Input: part model. Units: mm. Frame: model coordinates. A direction names the side the tool comes from. Coordinates: 2 decimals unless noted, no trailing zeros. Write each loop counter-clockwise with the first axis right and the second up, starting at its lowest first coordinate (ties: lowest second). Pieces come first, ordered by that corner, then holes. Notation, with made-up numbers: (77, 28) - (86, 28) arc R22 ccw to (86, 46) - close; hole circle Ø4 at (-15.75, 7.5). An arc over 180 degrees is marked (long way). Use CSV: the item, a comma, the result in double quotes.
```python
from build123d import *

# Parameters (mm, degrees)
CHAMFER1_SIZE      = 3
SKETCH2_W          = 4
SKETCH2_H          = 70.381112312
CUT_EXTRUDE2_DEPTH = 228.158534949


with BuildPart() as part:
    # Sketch1 → Revolve1 (revolve)
    with BuildSketch(Plane.XY, mode=Mode.PRIVATE) as revolve1_sk:
        Polygon((0, 115), (36, 115), (36, 112), (51, 112), (51, 120), (151, 120), (151, 103.5), (36, 98.7), (0, 98.7), align=None)
    revolve(revolve1_sk.sketch.rotate(Axis((0, 0, 0), (1, 0, 0)), 90), axis=Axis((0, 0, 0), (1, 0, 0)))

    # Chamfer1
    chamfer1_edges = [part.edges().sort_by_distance(p)[0] for p in [
        (0, 0, -115),
    ]]
    chamfer(chamfer1_edges, length=CHAMFER1_SIZE)

    # Sketch2 → Cut-Extrude2 (cut, through all)
    with BuildSketch(Plane(origin=(0, 0, 0), x_dir=(0, 0, -1), z_dir=(1, 0, 0))):
        with Locations((0, 103.5)):
            Rectangle(SKETCH2_W, SKETCH2_H)
    extrude(amount=CUT_EXTRUDE2_DEPTH, mode=Mode.SUBTRACT)


solid = part.part
```
(1) Draft query along Z for faces 1 (the flat face through (36, 110, 25)), 2 (the flat face through (74, 109, 2)). Return one class per face: pulls with the +Z half, pulls with the -Z half, needs draft (parallel to the pull), parting line crosses it, or undercut.
Check values:
face 1,"needs draft"
face 2,"undercut"
(2) Reachability of faces 3 (the flat face through (74, 109, -2)), 4 (the flat face through (51, -107, -35)), 5 (the flat face through (151, -89, -54)) from +Z, -Z, +X, -X, +Y, -Y: full face, straight path, thin tool, end or side. Return the list, or none.
Check values:
face 3,"+X, -X, +Y"
face 4,"none"
face 5,"+Z, -Z, +X, +Y, -Y"
(3) Ray query, probe 1 along Z at (x, y) = (142, 87.5); probe 2 along Y at (x, z) = (9, 0); probe 3 along Z at (x, y) = (135.5, 17.5). Return the intervals inside material, ascending. Write a range as from..to.
Check values:
probe 1,"-82.12..-54.57, 54.57..82.12"
probe 2,"-115..-98.7"
probe 3,"-118.72..-101.35, 101.35..118.72"
(4) Pin query (flat end, axial travel): pin 1 Ø6 at (x, y) = (33.5, 88) entering from -Z; pin 2 Ø23.5 at (x, y) = (82, 109) entering from -Z; pin 3 Ø2 at (x, y) = (32, 54) entering from -Z. Return the tip coordinate at first contact, or that it passes through.
Check values:
pin 1,"z = -77.46"
pin 2,"z = -70.3"
pin 3,"z = -102.06"
(5) Cut plane B-B on x = 60. Return loops of the section in (y, z), and give its area (3 significant figures).
Check values:
outline,"(99.68, -2) arc R99.7 cw (long way) to (99.68, 2) - (119.98, 2) arc R120 ccw (long way) to (119.98, -2) - close"
area,"13,900 mm^2"
(6) Cut plane A-A on x = 139. Return loops of the section in (y, z), and give its area (3 significant figures).
Check values:
outline,"(102.98, -2) arc R103 cw (long way) to (102.98, 2) - (119.98, 2) arc R120 ccw (long way) to (119.98, -2) - close"
area,"11,800 mm^2"
